from build123d import *

# Parameters (mm, degrees)
SKETCH1_R           = 5
BOSS_EXTRUDE1_DEPTH = 5


with BuildPart() as part:
    # Sketch1 → Boss-Extrude1 (new body)
    with BuildSketch(Plane.XY):
        with BuildLine():
            Line((9.797958971, 5), (40.202041029, 5))
            ThreePointArc((40.202041029, 5), (42.091863394, 5.370899501), (43.70131209, 6.428571429))
            ThreePointArc((43.70131209, 6.428571429), (59, 0), (43.70131209, -6.428571429))
            ThreePointArc((43.70131209, -6.428571429), (42.091863394, -5.370899501), (40.202041029, -5))
            Line((40.202041029, -5), (9.797958971, -5))
            ThreePointArc((9.797958971, -5), (7.908136606, -5.370899501), (6.29868791, -6.428571429))
            ThreePointArc((6.29868791, -6.428571429), (-9, 0), (6.29868791, 6.428571429))
            ThreePointArc((6.29868791, 6.428571429), (7.908136606, 5.370899501), (9.797958971, 5))
        make_face()
        Circle(SKETCH1_R, mode=Mode.SUBTRACT)
        with Locations((50, 0)):
            Circle(SKETCH1_R, mode=Mode.SUBTRACT)
    extrude(amount=BOSS_EXTRUDE1_DEPTH)


solid = part.part
The listing builds one solid part. Answer for the finished solid, in the listing's coordinates (mm). A direction names the side the tool comes from. Give positions to 0.01 mm unless a question says otherwise; leave off trailing zeros. Loops run counter-clockwise (first coordinate to the right, second up) from the corner with the lowest first, then second, coordinate; pieces in that order, holes last.
Item 1: A cutting plane is placed at D-D (y = 0). Give the vertices of the cut face in (x, z), then the cut area to 3 significant figures.
Derived:
outline: (-9, 0) - (-5, 0) - (-5, 5) - (-9, 5) - close; (5, 0) - (45, 0) - (45, 5) - (5, 5) - close; (55, 0) - (59, 0) - (59, 5) - (55, 5) - close
area: 240 mm2
Item 2: A tool of negligible diameter and unlimited length cuts with its end or side. For faces 1 (the flat face through (25, 0, 0)), 2 (the cylindrical face through (42.07, 5.36, 2.46)), 3 (the flat face through (25, -5, 2)), from which of +Z, -Z, +X, -X, +Y, -Y can it reach the whole face along a straight path? Write none if from no direction.
Derived:
face 1: -Z, +X, -X, +Y, -Y
face 2: +Z, -Z, +Y
face 3: +Z, -Z, -Y
Item 3: A cutting plane is placed at C-C (z = 3.45). Give the vertices of the cut face in (x, y), then the cut area to 3 significant figures.
Derived:
outline: (6.3, -6.43) arc R5 cw to (9.8, -5) - (40.2, -5) arc R5 cw to (43.7, -6.43) arc R9 ccw (long way) to (43.7, 6.43) arc R5 cw to (40.2, 5) - (9.8, 5) arc R5 cw to (6.3, 6.43) arc R9 ccw (long way) to start; hole circle Ø10 at (0, 0); hole circle Ø10 at (50, 0)
area: 684 mm2
Item 4: A cutting plane is placed at A-A (x = 50). Give the vertices of the cut face in (y, z), then the cut area to 3 significant figures.
Derived:
outline: (-9, 0) - (-5, 0) - (-5, 5) - (-9, 5) - close; (5, 0) - (9, 0) - (9, 5) - (5, 5) - close
area: 40.0 mm2
Item 5: Determine the mould class of faces 4 (the cylindrical face through (42.117, -5.381, 2.465)), 5 (the flat face through (25, 0, 5)) for opening direction X: +X half, -X half, draft (parallel to the pull), parting line (faces both ways), or undercut.
Derived:
face 4: undercut
face 5: draft
Item 6: Each of these flat-tipped pins is pushed along its axis until it touches: pin 1 Ø1 at (x, z) = (39, 2) entering from -Y; pin 2 Ø2 at (y, z) = (3, 4.5) entering from +X; pin 3 Ø3 at (y, z) = (6, 2) entering from -X. Where does it stop, or does it pass through?
Derived:
pin 1: stops at y = -5
pin 2: stops at x = 58.77
pin 3: stops at x = -7.79
Item 7: Find the intervals of material crossed by line 1 along Y through (x, z) = (0, 2.75); line 2 along X through (y, z) = (2.5, 4.2); line 3 along X through (y, z) = (-4.5, 0.4), in increasing order.
Derived:
line 1: y = -9 to -5, 5 to 9
line 2: x = -8.65 to -4.33, 4.33 to 45.67, 54.33 to 58.65
line 3: x = -7.79 to -2.18, 2.18 to 47.82, 52.18 to 57.79
Item 8: A cutting plane is placed at B-B (y = 7.25). Give the vertices of the cut face in (x, z), then the cut area to 3 significant figures.
Derived:
outline: (-5.33, 0) - (5.33, 0) - (5.33, 5) - (-5.33, 5) - close; (44.67, 0) - (55.33, 0) - (55.33, 5) - (44.67, 5) - close
area: 107 mm2
